Geometry check sheet. Reference: drawing and pictorial views, mm from the part's lowest x, y, z. A direction names the side the tool comes from. Give positions to 0.01 mm unless a question says otherwise; leave off trailing zeros. Order: outer loops, then holes, each group sorted by start corner. A loop starts at its lowest first (then second) coordinate and runs counter-clockwise, first axis right, second up. Notation, with made-up numbers: (-12.5, 43.25) -> (18.5, 43.25) arc R10 cw to (18.5, 56.25) -> close; hole circle Ø5 at (66, 73). An arc over 180 degrees is marked (long way). Write each question's results on one line, items separated by ' | '.
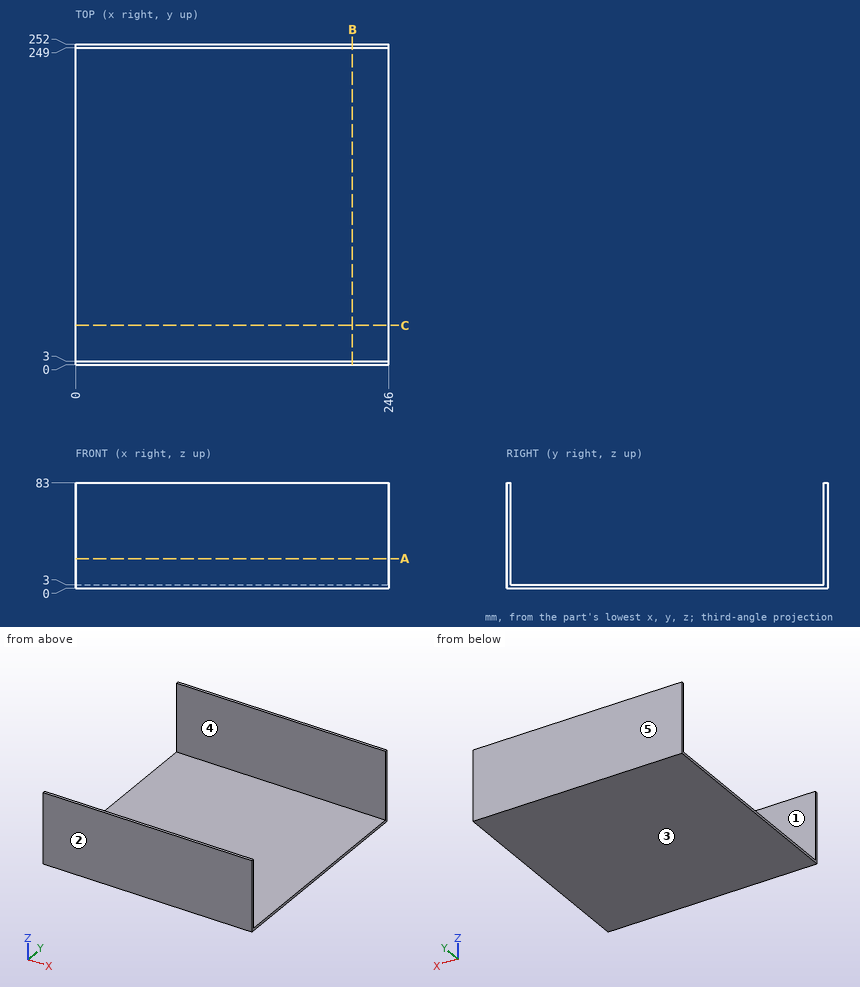
1. Access from +Z, -Z, +X, -X, +Y, -Y to the whole of each face (thin tool, end or side, straight path). Record for the marked faces 4 and 5.
Verdict:
face 4: +Z, +X, -X | face 5: +Z, -Z, +X, -X, +Y
2. Gauge pin test, flat ends, axial feed: pin 1 Ø1.5 at (x, y) = (136.5, 166.5) entering from +Z; pin 2 Ø2 at (x, z) = (142, 8.5) entering from -Y. Record the tip position at first contact, or that the pin passes through.
Verdict:
pin 1: stops at z = 3 | pin 2: stops at y = 0
3. Mould release check, pull along Y, two halves, no side actions. Record for the marked faces 1, 2 and 3: +Y half, -Y half, draft (parallel to the pull), parting line (faces both ways), or undercut.
Verdict:
face 1: undercut | face 2: -Y half | face 3: draft
4. Material ranges on probe 1 along Y at (x, z) = (30, 62); probe 2 along Z at (x, y) = (28, 134), recorded low to high. Write a range as from..to.
Verdict:
probe 1: y = 0..3, 249..252 | probe 2: z = 0..3
5. Section check B-B on x = 217.5. Record the cut outline in (y, z), then the cut area to 3 significant figures.
Verdict:
outline: (0, 0) -> (252, 0) -> (252, 83) -> (249, 83) -> (249, 3) -> (3, 3) -> (3, 83) -> (0, 83) -> close | area: 1,240 mm^2
6. Section check C-C on y = 31. Record the cut outline in (x, z).
Verdict:
outline: (0, 0) -> (246, 0) -> (246, 3) -> (0, 3) -> close
7. Section check A-A on z = 23.5. Record the cut outline in (x, y), then the cut area to 3 significant figures.
Verdict:
outline: (0, 0) -> (246, 0) -> (246, 3) -> (0, 3) -> close; (0, 249) -> (246, 249) -> (246, 252) -> (0, 252) -> close | area: 1,480 mm^2
